from build123d import *

# Parameters (mm, degrees)
CLEVIS_PROFILE_SKETCH_R = 7.5
CLEVIS_BODY_DEPTH       = 21.5
CLEVIS_GAP_SKETCH_W     = 27
CLEVIS_GAP_SKETCH_H     = 45
CLEVIS_GAP_CUT_DEPTH    = 186.5


with BuildPart() as part:
    # Clevis Profile Sketch → Clevis Body (new, symmetric)
    with BuildSketch(Plane.XY):
        with BuildLine():
            ThreePointArc((-34, -14.857864376), (-33.619397663, -12.944447214), (-32.535533906, -11.32233047))
            Line((-32.535533906, -11.32233047), (-10.606601718, 10.606601718))
            ThreePointArc((-10.606601718, 10.606601718), (-3.851711358, 14.497045203), (3.943382345, 14.47237837))
            Line((3.943382345, 14.47237837), (87.314460782, -8.24427748))
            ThreePointArc((87.314460782, -8.24427748), (89.973179074, -10.032971502), (91, -13.068403604))
            Line((91, -13.068403604), (91, -22))
            Line((91, -22), (85, -22))
            Line((85, -22), (85, -40))
            Line((85, -40), (-28, -40))
            Line((-28, -40), (-28, -22))
            Line((-28, -22), (-34, -22))
            Line((-34, -22), (-34, -14.857864376))
        make_face()
        Circle(CLEVIS_PROFILE_SKETCH_R, mode=Mode.SUBTRACT)
    extrude(amount=CLEVIS_BODY_DEPTH, both=True)

    # Clevis Gap Sketch → Clevis Gap Cut (cut, symmetric)
    with BuildSketch(Plane(origin=(85, 0, 0), x_dir=(0, 0, -1), z_dir=(1, 0, 0))):
        with Locations((0, -7.5)):
            Rectangle(CLEVIS_GAP_SKETCH_W, CLEVIS_GAP_SKETCH_H)
        with BuildLine():
            Line((-21.5, -40), (21.5, -40))
            ThreePointArc((21.5, -40), (0, -38.548888359), (-21.5, -40))
        make_face()
    extrude(amount=CLEVIS_GAP_CUT_DEPTH, both=True, mode=Mode.SUBTRACT)


solid = part.part
Model file for the job. Use its own axes, mm. A direction names the side the tool comes from. Round coordinates to 2 decimals unless told otherwise and drop trailing zeros. Loops run counter-clockwise (first coordinate to the right, second up) from the corner with the lowest first, then second, coordinate; pieces in that order, holes last. Notation, with made-up numbers: (40, 67) -> (52, 67) arc R23 ccw to (52, 104) -> close; hole circle Ø2 at (-34, 59). An arc over 180 degrees is marked (long way). Answer as CSV lines item,"result". Start each with the question number.
1) Slice it at D-D (z = -18). List the corners of the cut face in (x, y).
2) Tool access for faces 1 (the face through (91, -17, 18)), 2 (the face through (-31, -22, 18)), 3 (the face through (88, -22, -17)): list every direction of +Z, -Z, +X, -X, +Y, -Y with a clear straight run to the whole face (end or side of a thin tool).
3) Pin check, flat tips, straight feed: P1, Ø1.8, axis at x = 88, z = -16, coming from the -Y side; P2, Ø6.5, axis at x = -31, z = 19.5, coming from the -Y side; P3, Ø13.5, axis at x = 0, y = 0, coming from the -Z side; P4, Ø13.5, axis at x = 3.5, z = 3.5, coming from the +Y side. Stop position of each tip, or through.
4) Slice it at B-B (x = 0). List the corners of the cut face in (y, z).
5) Slice it at C-C (y = 0). List the corners of the cut face in (x, z).
6) Mould opens along Z. For faces 4 (the face through (28, -13, -13.5)), 5 (the face through (-3.958, 14.468, -17.444)), 6 (the face through (28, -30, 0)), 7 (the face through (29, -18, 21.5)) say: +Z half, -Z half, draft (parallel to the pull), parting line (faces both ways), or undercut.
7) Probe line 1 along Z through (x, y) = (51, -9.5); line 2 along X through (y, z) = (-29.5, 18.5); line 3 along Y through (x, z) = (0, -18.5). List the from-to ranges inside material, lowest first.
8) Slice it at A-A (y = -20.5). List the corners of the cut face in (x, z), plus the area to 3 significant figures.
Filled in:
1,outline,"(-34, -22) -> (-28, -22) -> (-28, -39.56) -> (85, -39.56) -> (85, -22) -> (91, -22) -> (91, -13.07) arc R5 ccw to (87.31, -8.24) -> (3.94, 14.47) arc R15 ccw to (-10.61, 10.61) -> (-32.54, -11.32) arc R5 ccw to (-34, -14.86) -> close; hole circle Ø15 at (0, 0)"
2,face 1,"+Z, -Z, +X, +Y, -Y"
2,face 2,"+Z, -Z, -X, -Y"
2,face 3,"+Z, -Z, +X, -Y"
3,P1,"stops at y = -22"
3,P2,"stops at y = -39.9"
3,P3,"passes through"
3,P4,"stops at y = -30"
4,outline,"(-40, -21.5) -> (-7.5, -21.5) -> (-7.5, -13.5) -> (-30, -13.5) -> (-30, 13.5) -> (-7.5, 13.5) -> (-7.5, 21.5) -> (-40, 21.5) arc R160 cw to start; (7.5, -21.5) -> (15, -21.5) -> (15, -13.5) -> (7.5, -13.5) -> close; (7.5, 13.5) -> (15, 13.5) -> (15, 21.5) -> (7.5, 21.5) -> close"
5,outline,"(-21.21, -21.5) -> (-7.5, -21.5) -> (-7.5, -13.5) -> (-21.21, -13.5) -> close; (-21.21, 13.5) -> (-7.5, 13.5) -> (-7.5, 21.5) -> (-21.21, 21.5) -> close; (7.5, -21.5) -> (57.06, -21.5) -> (57.06, -13.5) -> (7.5, -13.5) -> close; (7.5, 13.5) -> (57.06, 13.5) -> (57.06, 21.5) -> (7.5, 21.5) -> close"
6,face 4,"undercut"
6,face 5,"draft"
6,face 6,"undercut"
6,face 7,"+Z half"
7,line 1,"z = -21.5 to -13.5, 13.5 to 21.5"
7,line 2,"x = -28 to 85"
7,line 3,"y = -39.62 to -7.5, 7.5 to 15"
8,outline,"(-34, -21.5) -> (91, -21.5) -> (91, -13.5) -> (-34, -13.5) -> close; (-34, 13.5) -> (91, 13.5) -> (91, 21.5) -> (-34, 21.5) -> close"
8,area,"2,000 mm2"
